Source: CAD feature listing. Evaluate the final solid. Frame: model axes, mm. Give positions to 0.01 mm unless a question says otherwise; leave off trailing zeros. Loops run counter-clockwise (first coordinate to the right, second up) from the corner with the lowest first, then second, coordinate; pieces in that order, holes last.
```python
from build123d import *

# Parameters (mm, degrees)
EXTRUDE_2_DEPTH = 8


with BuildPart() as part:
    # 草图1 → 凸台-拉伸2 (new body)
    with BuildSketch(Plane.XY):
        with BuildLine():
            Line((330, 0), (30, 0))
            Line((30, 0), (30, -19.046909383))
            ThreePointArc((30, -19.046909383), (35.404988471, -36.22495956), (49.672360525, -47.213198859))
            Line((49.672360525, -47.213198859), (330, -150))
            Line((330, -150), (330, 0))
        make_face()
    extrude(amount=EXTRUDE_2_DEPTH)


solid = part.part
```
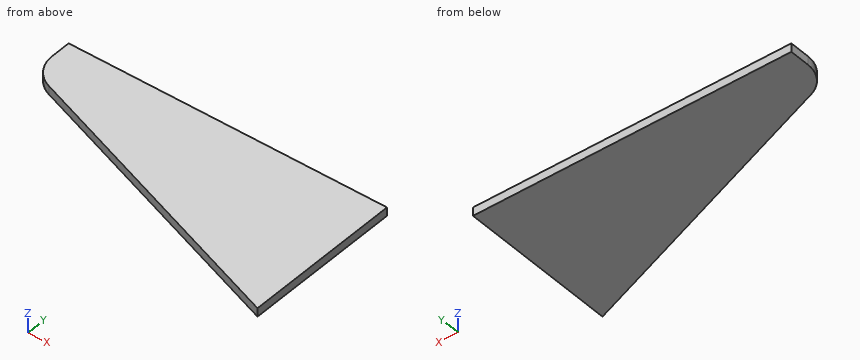
(1) First-contact query: pin 1 (1 mm diameter, centred on x = 181.5, z = 5, fed in from -Y); pin 2 (3 mm diameter, centred on x = 171, z = 3, fed in from -Y). Flat tips, straight axial feed; report the tip coordinate or a pass-through.
A:
pin 1: stops at y = -95.73
pin 2: stops at y = -92.25
(2) Ray query, line 1 along Y through (x, z) = (297, 2.25); line 2 along Y through (x, z) = (251, 4.25); line 3 along X through (y, z) = (-44, 0.75). Return the intervals inside material, ascending.
A:
line 1: y = -137.9 to 0
line 2: y = -121.03 to 0
line 3: x = 43.35 to 330
(3) Section B-B, the plane x = 220.5. Return the cut outline in (y, z).
A:
outline: (-109.85, 0) - (0, 0) - (0, 8) - (-109.85, 8) - close
(4) Section A-A, the plane z = 3.25. Return the cut outline in (x, y), then the cut area to 3 significant figures.
A:
outline: (30, -19.05) arc R30 ccw to (49.67, -47.21) - (330, -150) - (330, 0) - (30, 0) - close
area: 28,400 mm2
(5) Section C-C, the plane y = -99. Return the cut outline in (x, z), then the cut area to 3 significant figures.
A:
outline: (190.91, 0) - (330, 0) - (330, 8) - (190.91, 8) - close
area: 1,110 mm2
